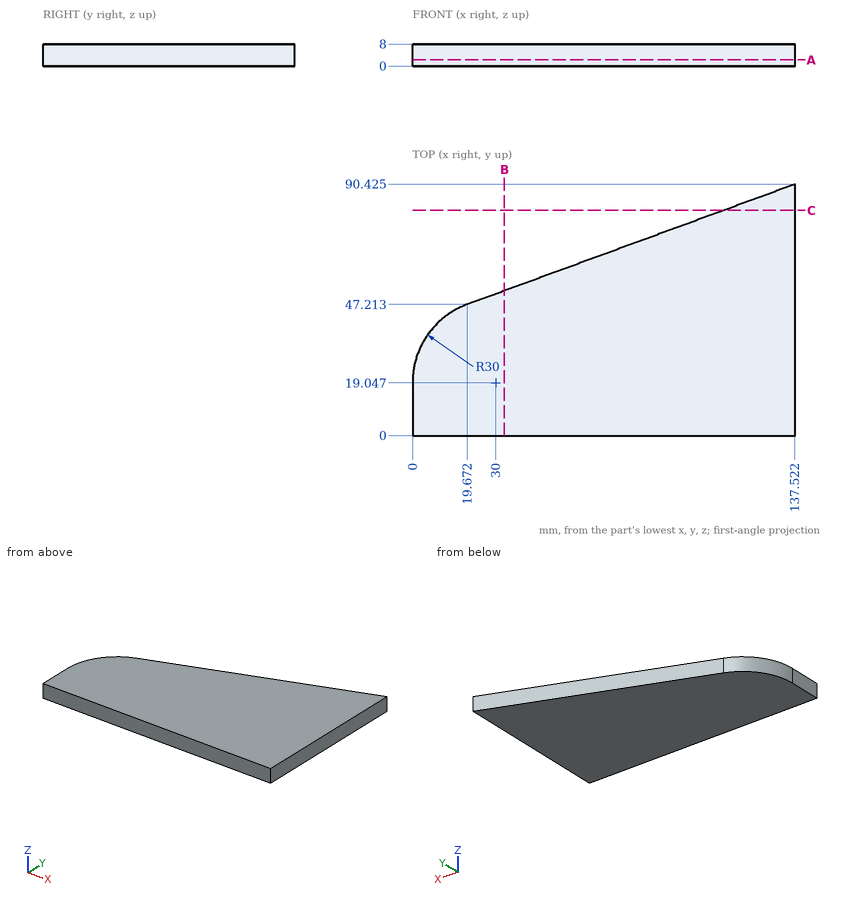
Print and shaded views of the part. All mm, measured from the part's lowest x, y and z. Coordinates: 2 decimals unless noted, no trailing zeros. Order: outer loops, then holes, each group sorted by start corner. A loop starts at its lowest first (then second) coordinate and runs counter-clockwise, first axis right, second up. Notation, with made-up numbers: M 16,-3 L 68,-3 A21 ccw 68,22 Z; hole C 71.25,24.25 d6. An arc over 180 degrees is marked long. Write each question's results on one line, items separated by ' | '. Start each with the question number.
Q1. Cut at A-A (z = 2.25). List the corners of the cut face in (x, y) (1 decimal), then the cut area to 3 significant figures.
Q2. Drill centre lines: probe 1 along Y at (x, z) = (47, 1.75); probe 2 along Y at (x, z) = (76, 1.75); probe 3 along X at (y, z) = (23, 3). Where is each one in solid material? Low to high. Write a range as from..to.
Q3. Cut at C-C (y = 81). List the corners of the cut face in (x, z).
Q4. Flat gauge pin, fed straight in: P1, Ø1.5, axis at x = 108, z = 7, coming from the +Y side (1 decimal). Where does the tip first touch, or does it go through?
Q5. Cut at B-B (x = 33). List the corners of the cut face in (y, z), then the cut area to 3 significant figures.
Found:
1) outline: M 0,0 L 137.5,0 L 137.5,90.4 L 19.7,47.2 A30 ccw 0,19 Z | area: 8,890 mm²
2) probe 1: 0..57.23 | probe 2: 0..67.87 | probe 3: 0.26..137.52
3) outline: M 111.82,0 L 137.52,0 L 137.52,8 L 111.82,8 Z
4) P1: y = 79.9
5) outline: M 0,0 L 52.1,0 L 52.1,8 L 0,8 Z | area: 417 mm²
